from build123d import *

# Parameters (mm, degrees)
BARREL_AND_PLATE_PROFILE_SKETCH_R = 3
BARREL_AND_PLATE_70MM_DEPTH       = 70
PLATE_PROFILE_TRIM_DEPTH          = 70
LOWER_PLATE_DEPTH                 = 63
KEYHOLE_CUT_DEPTH                 = 63
KEYHOLE_CUT_DEPTH_BACK            = 63
KEYHOLE_SKETCH_W                  = 3.828036988
KEYHOLE_SKETCH_H                  = 46.115634491
KEYHOLE_SKETCH_W_2                = 17.383946001
CORNER_CHAMFER_CUT_DEPTH          = 63
CORNER_CHAMFER_CUT_DEPTH_BACK     = 63
CORNER_CHAMFER_SKETCH_W           = 7.615823962
CORNER_CHAMFER_SKETCH_H           = 47.440125615
CURVED_LOWER_EDGE_CUT_DEPTH       = 63
CURVED_LOWER_EDGE_CUT_DEPTH_BACK  = 63


with BuildPart() as part:
    # Barrel and Plate Profile Sketch → Barrel and Plate 70mm (new body)
    with BuildSketch(Plane(origin=(0, 0, 0), x_dir=(0, 0, -1), z_dir=(1, 0, 0))):
        with BuildLine():
            Line((-2.5, -5.454356057), (-2.5, -38))
            Line((-2.5, -38), (2.5, -38))
            Line((2.5, -38), (2.5, -5.454356057))
            ThreePointArc((2.5, -5.454356057), (0, 6), (-2.5, -5.454356057))
        make_face()
        Circle(BARREL_AND_PLATE_PROFILE_SKETCH_R, mode=Mode.SUBTRACT)
    extrude(amount=BARREL_AND_PLATE_70MM_DEPTH)

    # Plate Profile Trim Sketch → Plate Profile Trim (cut)
    with BuildSketch(Plane(origin=(0, 0, -2.5), x_dir=(-1, 0, 0), z_dir=(0, 0, -1))):
        with BuildLine():
            Line((-70, -28.297812678), (-70, -38))
            Line((-70, -38), (-61.208453248, -38))
            ThreePointArc((-61.208453248, -38), (-66.50641986, -33.966420344), (-70, -28.297812678))
        make_face()
        with BuildLine():
            Line((-7.077917117, -38), (0, -38))
            Line((0, -38), (0, -28.297812678))
            ThreePointArc((0, -28.297812678), (-3.407881829, -33.244529129), (-7.077917117, -38))
        make_face()
    extrude(amount=-PLATE_PROFILE_TRIM_DEPTH, mode=Mode.SUBTRACT)

    # Lower Plate Sketch → Lower Plate (add)
    with BuildSketch(Plane(origin=(70, 0, 0), x_dir=(0, 0, -1), z_dir=(1, 0, 0))):
        with BuildLine():
            Line((5.265785985, -82.841381432), (10.265785985, -82.324852713))
            ThreePointArc((10.265785985, -82.324852713), (-0.231731323, -61.32131925), (2.5, -38))
            Line((2.5, -38), (-2.5, -38))
            ThreePointArc((-2.5, -38), (-4.109661448, -61.371910347), (5.265785985, -82.841381432))
        make_face()
    extrude(amount=-LOWER_PLATE_DEPTH)

    # Keyhole Sketch → Keyhole Cut (cut, two sides: drawn at the far end of the back side and taken through both)
    with BuildSketch(Plane.XY.offset(-KEYHOLE_CUT_DEPTH_BACK)):
        with Locations((8.914018494, -61.057817246)):
            Rectangle(KEYHOLE_SKETCH_W, KEYHOLE_SKETCH_H)
        with Locations((61.572603173, -61.057817246)):
            Rectangle(KEYHOLE_SKETCH_W_2, KEYHOLE_SKETCH_H)
    extrude(amount=KEYHOLE_CUT_DEPTH + KEYHOLE_CUT_DEPTH_BACK, mode=Mode.SUBTRACT)

    # Corner Chamfer Sketch → Corner Chamfer Cut (cut, two sides: drawn at the far end of the back side and taken through both)
    with BuildSketch(Plane.XY.offset(-CORNER_CHAMFER_CUT_DEPTH_BACK)):
        with Locations((12.649212284, -61.720062807)):
            Rectangle(CORNER_CHAMFER_SKETCH_W, CORNER_CHAMFER_SKETCH_H)
    extrude(amount=CORNER_CHAMFER_CUT_DEPTH + CORNER_CHAMFER_CUT_DEPTH_BACK, mode=Mode.SUBTRACT)

    # Curved Lower Edge Sketch → Curved Lower Edge Cut (cut, two sides: drawn at the far end of the back side and taken through both)
    with BuildSketch(Plane(origin=(0, 0, -2.5), x_dir=(-1, 0, 0), z_dir=(0, 0, -1)).offset(-CURVED_LOWER_EDGE_CUT_DEPTH_BACK)):
        with BuildLine():
            Line((-42.377724671, -51.285597096), (-42.400406488, -51.831163346))
            ThreePointArc((-42.400406488, -51.831163346), (-35.827806952, -58.403762881), (-29.255207417, -51.831163346))
            Line((-29.255207417, -51.831163346), (-29.255207417, -38))
            Line((-29.255207417, -38), (-41.825378407, -38))
            Line((-41.825378407, -38), (-42.377724671, -51.285597096))
        make_face()
        with BuildLine():
            ThreePointArc((-29.255207417, -37.597568213), (-36.178737372, -17.856631692), (-41.825378407, -38))
            Line((-41.825378407, -38), (-29.255207417, -38))
            Line((-29.255207417, -38), (-29.255207417, -37.597568213))
        make_face()
    extrude(amount=CURVED_LOWER_EDGE_CUT_DEPTH + CURVED_LOWER_EDGE_CUT_DEPTH_BACK, mode=Mode.SUBTRACT)


solid = part.part
Input: part model. Units: mm. Frame: model coordinates. A direction names the side the tool comes from. Give positions to 0.01 mm unless a question says otherwise; leave off trailing zeros. Write each loop counter-clockwise with the first axis right and the second up, starting at its lowest first coordinate (ties: lowest second). Pieces come first, ordered by that corner, then holes. Notation, with made-up numbers: (58, 79.25) -> (98, 79.25) arc R20 cw to (98, 106.25) -> close; hole circle Ø6 at (52.25, -35). An arc over 180 degrees is marked (long way). Use one line per item in the form item = value. Start each with the question number.
1) Section query D-D on x = 33.5. Return the cut outline in (y, z).
2) Section query B-B on z = -0.75. Return the cut outline in (x, y).
3) Draft query along Y for faces 6 (the flat face through (0, -7, 0)), 7 (the cylindrical face through (35, 0, 3)), 8 (the flat face through (12, -38, 0)). Return one class per face: pulls with the +Y half, pulls with the -Y half, needs draft (parallel to the pull), parting line crosses it, or undercut.
4) Ray query, probe 1 along Z at (x, y) = (6.5, -17.5); probe 2 along Y at (x, z) = (33.5, 1); probe 3 along Y at (x, z) = (56.5, -2.25). Return the intervals inside material, ascending. Write a range as from..to.
5) Set-up query: faces 1 (the cylindrical face through (36, -58.4, 2.8)), 2 (the flat face through (35, -14, 2.5)), 3 (the flat face through (35, -15, -2.5)), 4 (the flat face through (52.881, -61, 1)), 5 (the flat face through (16.457, -61, 1)). Return all of +Z, -Z, +X, -X, +Y, -Y with unobstructed straight access to the full face (end or side cutting, diameter ignored); none if empty.
6) Section query A-A on y = 0. Return the cut outline in (x, z).
7) Pin query (flat end, axial travel): pin 1 (10 mm diameter, centred on x = 37.5, y = -16.5, fed in from +Z); pin 2 (4 mm diameter, centred on x = 19.5, z = -6, fed in from +Y); pin 3 (3 mm diameter, centred on x = 41, z = -7, fed in from +Y); pin 4 (13 mm diameter, centred on x = 35.83, y = -28.82, fed in from -Z). Return the tip coordinate at first contact, or that it passes through.
8) Section query C-C on x = 9.5. Return the cut outline in (y, z).
Outcome:
q1.outline = (-82.84, -5.27) -> (-82.32, -10.27) arc R41.05 cw to (-57.98, 0.68) -> (-57.98, 4.58) arc R49.23 ccw to start; (-18.1, -2.5) -> (-5.45, -2.5) arc R6 ccw (long way) to (-5.45, 2.5) -> (-18.1, 2.5) -> close; hole circle Ø6 at (0, 0)
q2.outline = (0, -28.3) arc R111.2 ccw to (7.08, -38) -> (16.46, -38) -> (16.46, -42.9) -> (29.26, -42.9) -> (29.26, -37.6) arc R10.97 cw (long way) to (41.83, -38) -> (42.03, -42.9) -> (52.88, -42.9) -> (52.88, -38) -> (61.21, -38) arc R18.21 ccw to (70, -28.3) -> (70, -2.9) -> (0, -2.9) -> close; (0, 2.9) -> (70, 2.9) -> (70, 5.95) -> (0, 5.95) -> close; (16.46, -75.74) -> (52.88, -75.74) -> (52.88, -65.58) -> (16.46, -65.58) -> close
q3.face_6 = needs draft
q3.face_7 = undercut
q3.face_8 = pulls with the -Y half
q4.probe_1 = -2.5..2.5
q4.probe_2 = -72.01..-57.98, -18.1..-2.83, 2.83..5.92
q4.probe_3 = -38..-1.98, 1.98..5.56
q5.face_1 = +Z, -Z
q5.face_2 = +Z, +X, -X
q5.face_3 = -Z, +X, -X
q5.face_4 = +Z, -Z, +X, -Y
q5.face_5 = +Z, -Z, -X, -Y
q6.outline = (0, -6) -> (70, -6) -> (70, -3) -> (0, -3) -> close; (0, 3) -> (70, 3) -> (70, 6) -> (0, 6) -> close
q7.pin_1 = 2.5
q7.pin_2 = 4.47
q7.pin_3 = 2.4
q7.pin_4 = through
q8.outline = (-38, -2.5) -> (-5.45, -2.5) arc R6 ccw (long way) to (-5.45, 2.5) -> (-38, 2.5) -> close; hole circle Ø6 at (0, 0)
